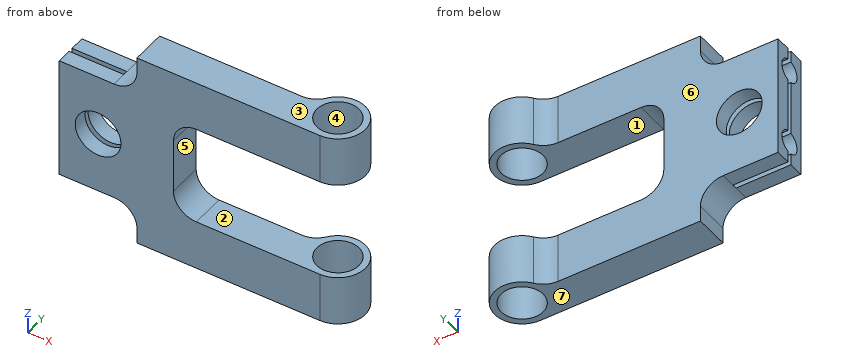
```python
from build123d import *

# Parameters (mm, degrees)
BASE_PLATE_SKETCH_R     = 10
BASE_PLATE_DEPTH        = 7.5
KNUCKLE_A_SKETCH_R      = 12
KNUCKLE_A_SKETCH_R_2    = 9
KNUCKLE_A_DEPTH         = 22
KNUCKLE_A_BORE_SKETCH_R = 9.21075175
KNUCKLE_A_BORE_DEPTH    = 22
KNUCKLE_A_BLEND_R10_R   = 10
KNUCKLE_START           = -22
KNUCKLE_B_SKETCH_R      = 12
KNUCKLE_B_SKETCH_R_2    = 9.21075175
KNUCKLE_B_DEPTH         = 22
KNUCKLE_B_BORE_SKETCH_R = 9.21075175
KNUCKLE_B_BORE_DEPTH    = 22
KNUCKLE_B_BLEND_R10_R   = 10
GROOVE_CUT_SKETCH_W     = 54
GROOVE_CUT_SKETCH_H     = 2
GROOVE_CUT_DEPTH        = 32
HOLE_CUT_SKETCH_R       = 5
HOLE_CUT_DEPTH          = 34


with BuildPart() as part:
    # Base Plate Sketch → Base Plate (new, symmetric)
    with BuildSketch(Plane(origin=(0, 0, 0), x_dir=(1, 0, 0), z_dir=(0, 1, 0))):
        with BuildLine():
            Line((0, 44), (0, 22))
            Line((0, 22), (-54, 22))
            ThreePointArc((-54, 22), (-61.071067812, 19.071067812), (-64, 12))
            Line((-64, 12), (-64, -12))
            ThreePointArc((-64, -12), (-61.071067812, -19.071067812), (-54, -22))
            Line((-54, -22), (0, -22))
            Line((0, -22), (0, -44))
            Line((0, -44), (-64, -44))
            Line((-64, -44), (-80, -44))
            Line((-80, -44), (-80, -37))
            ThreePointArc((-80, -37), (-82.928932188, -29.928932188), (-90, -27))
            Line((-90, -27), (-114, -27))
            Line((-114, -27), (-114, 27))
            Line((-114, 27), (-90, 27))
            ThreePointArc((-90, 27), (-82.928932188, 29.928932188), (-80, 37))
            Line((-80, 37), (-80, 44))
            Line((-80, 44), (-64, 44))
            Line((-64, 44), (0, 44))
        make_face()
        with Locations(Location((-97, 0, 0), (0, 0, 270))):
            Circle(BASE_PLATE_SKETCH_R, mode=Mode.SUBTRACT)
    extrude(amount=BASE_PLATE_DEPTH, both=True)

    # Knuckle A Sketch → Knuckle A (add)
    with BuildSketch(Plane.XY.offset(44)):
        with Locations((0, 4.5)):
            Circle(KNUCKLE_A_SKETCH_R)
        with Locations((0, 4.5)):
            Circle(KNUCKLE_A_SKETCH_R_2, mode=Mode.SUBTRACT)
    extrude(amount=-KNUCKLE_A_DEPTH)

    # Knuckle A Bore Sketch → Knuckle A Bore (cut)
    with BuildSketch(Plane.XY.offset(44)):
        with Locations((0, 4.5)):
            Circle(KNUCKLE_A_BORE_SKETCH_R)
    extrude(amount=-KNUCKLE_A_BORE_DEPTH, mode=Mode.SUBTRACT)

    # Knuckle A Blend R10
    knuckle_a_blend_r10_edges = [part.edges().sort_by_distance(p)[0] for p in [
        (-11.618950039, 7.5, 33),
    ]]
    fillet(knuckle_a_blend_r10_edges, radius=KNUCKLE_A_BLEND_R10_R)

    # Knuckle B Sketch → Knuckle B (add)
    with BuildSketch(Plane(origin=(0, 0, -44), x_dir=(-1, 0, 0), z_dir=(0, 0, -1)).offset(KNUCKLE_START)):
        with Locations((0, 4.5)):
            Circle(KNUCKLE_B_SKETCH_R)
        with Locations(Location((0, 4.5, 0), (0, 0, 180))):
            Circle(KNUCKLE_B_SKETCH_R_2, mode=Mode.SUBTRACT)
    extrude(amount=KNUCKLE_B_DEPTH)

    # Knuckle B Bore Sketch → Knuckle B Bore (cut)
    with BuildSketch(Plane(origin=(0, 0, -44), x_dir=(-1, 0, 0), z_dir=(0, 0, -1)).offset(KNUCKLE_START)):
        with Locations(Location((0, 4.5, 0), (0, 0, 180))):
            Circle(KNUCKLE_B_BORE_SKETCH_R)
    extrude(amount=KNUCKLE_B_BORE_DEPTH, mode=Mode.SUBTRACT)

    # Knuckle B Blend R10
    knuckle_b_blend_r10_edges = [part.edges().sort_by_distance(p)[0] for p in [
        (-11.618950039, 7.5, -33),
    ]]
    fillet(knuckle_b_blend_r10_edges, radius=KNUCKLE_B_BLEND_R10_R)

    # Groove Cut Sketch → Groove Cut (cut)
    with BuildSketch(Plane.ZY.offset(114)):
        Rectangle(GROOVE_CUT_SKETCH_W, GROOVE_CUT_SKETCH_H)
    extrude(amount=-GROOVE_CUT_DEPTH, mode=Mode.SUBTRACT)

    # Hole Cut Sketch → Hole Cut (cut)
    with BuildSketch(Plane.ZY.offset(114)):
        with Locations((-17, 0)):
            Circle(HOLE_CUT_SKETCH_R)
        with Locations((17, 0)):
            Circle(HOLE_CUT_SKETCH_R)
    extrude(amount=-HOLE_CUT_DEPTH, mode=Mode.SUBTRACT)


solid = part.part
```
Geometry: final body of the model. Coordinates: model frame, mm. Face numbers are marked on the shaded views. A direction names the side the tool comes from. Round coordinates to 2 decimals unless told otherwise and drop trailing zeros. Write each loop counter-clockwise with the first axis right and the second up, starting at its lowest first coordinate (ties: lowest second). Pieces come first, ordered by that corner, then holes.
Item 1: Mould query, pull axis Z, two halves, no side actions, for the marked faces 1, 2, 3 and 4. Classes: +Z half, -Z half, draft (parallel to the pull), parting line (faces both ways), or undercut.
Item 2: Material intervals for L1, parallel to Y at x = -101, z = -17; L2, parallel to Z at x = 3, y = -5.75; L3, parallel to Z at x = -97, y = 3.25, sorted ascending.
Item 3: Section query B-B (y = -3.25). Give the number of separate pieces and of enclosed holes in the cut face, plus the area to 3 significant figures.
Item 4: Pin query (flat end, axial travel): P1, Ø5, axis at x = -105.5, y = -4, coming from the -Z side; P2, Ø11, axis at x = 0, y = 4.5, coming from the +Z side; P3, Ø1.5, axis at x = -98.5, z = -25.5, coming from the +Y side; P4, Ø1, axis at y = 7, z = 33.5, coming from the -X side. Return the tip coordinate at first contact, or that it passes through.
Item 5: Set-up query: the marked faces 5, 6 and 7. Return all of +Z, -Z, +X, -X, +Y, -Y with unobstructed straight access to the full face (end or side cutting, diameter ignored); none if empty.
Item 6: Section query A-A (z = 0). Return loops of the section in (x, y), plus the area to 3 significant figures.
Item 7: Section query C-C (z = -13.5). Return loops of the section in (x, y), plus the area to 3 significant figures.
Completed:
1. face 1: undercut
1. face 2: undercut
1. face 3: +Z half
1. face 4: draft
2. L1: y = -7.5 to -5, 5 to 7.5
2. L2: z = -44 to -22, 22 to 44
2. L3: z = -27 to -20.8, -13.2 to -10, 10 to 13.2, 20.8 to 27
3. separate pieces: 3
3. enclosed holes: 1
3. area: 5,280 mm2
4. P1: stops at z = -27
4. P2: passes through
4. P3: stops at y = 7.5
4. P4: stops at x = -80.83
5. face 5: +X, +Y, -Y
5. face 6: +Z, -Z, -X, +Y
5. face 7: -Z, +X, -X, +Y, -Y
6. outline: (-114, -7.5) - (-107, -7.5) - (-107, -1) - (-114, -1) - close; (-114, 1) - (-107, 1) - (-107, 7.5) - (-114, 7.5) - close; (-87, -7.5) - (-64, -7.5) - (-64, 7.5) - (-87, 7.5) - (-87, 1) - (-82, 1) - (-82, -1) - (-87, -1) - close
6. area: 426 mm2
7. outline: (-114, -7.5) - (-63.89, -7.5) - (-63.89, 7.5) - (-114, 7.5) - (-114, 3.57) - (-80, 3.57) - (-80, -3.57) - (-114, -3.57) - close
7. area: 509 mm2
